Input: part model. Units: mm. Frame: model coordinates. A direction names the side the tool comes from. Coordinates: 2 decimals unless noted, no trailing zeros. Write each loop counter-clockwise with the first axis right and the second up, starting at its lowest first coordinate (ties: lowest second). Pieces come first, ordered by that corner, then holes. Notation, with made-up numbers: (82.25, 18.25) - (109.25, 18.25) arc R5 ccw to (109.25, 27.25) - close; hole circle Ø7 at (17, -23.5). An arc over 180 degrees is marked (long way). Put each result on its own line as item: value. Start each with the question number.
1. Cut plane B-B, the plane z = -3.25. Return loops of the section in (x, y).
2. Line query: line 1 (Z direction, x = 9, y = 6); line 2 (X direction, y = 0.25, z = -2.5); line 3 (Y direction, x = 8, z = 2.5). Output: solid intervals per line, ascending.
3. Access query for faces 1 (the cylindrical face through (10.29, -0.97, -8.66)), 2 (the cylindrical face through (-5.587, -0.975, 8.713)), 3 (the cylindrical face through (-0.09, -6.79, -5.79)), 4 (the flat face through (0, 0, -4.7)). Directions: +Z, -Z, +X, -X, +Y, -Y. A direction counts if a zero-diameter tool reaches every point of the face in a straight line with its end or side. Return the directions, or none.
4. Cut plane A-A, the plane x = 2.5. Return loops of the section in (y, z), and give its area (3 significant figures).
5. Cut plane C-C, the plane y = -6.25. Return loops of the section in (x, z).
6. Pull-direction query (X, two-part tool) for faces 5 (the cylindrical face through (0.09, 6.79, -5.79)), 6 (the flat face through (-8, 0, -10.9)); classes: released by +X, released by -X, zero draft, split by the parting line, or undercut.
7. Cut plane D-D, the plane y = 3.75. Return loops of the section in (x, z), and give its area (3 significant figures).
8. Pin query (flat end, axial travel): pin 1 (2 mm diameter, centred on y = -3.5, z = -3, fed in from -X); pin 2 (1.5 mm diameter, centred on x = 2.5, y = -0.5, fed in from -Z); pin 3 (3 mm diameter, centred on x = -12, z = -1, fed in from +Y). Return the tip coordinate at first contact, or that it passes through.
from build123d import *

# Parameters (mm, degrees)
SKETCH_2_R        = 5.08
EXTRUDE_1_DEPTH   = 4.7
EXTRUDE_1_2_DEPTH = 4.7
EXTRUDE_2_DEPTH   = 2.22
SKETCH_4_R        = 2.545
EXTRUDE_3_DEPTH   = 10.9
CHAMFER_1_SIZE    = 0.444


with BuildPart() as part:
    # Sketch 2 → Extrude 1 (new, symmetric)
    with BuildSketch(Plane.XY):
        with Locations((7.9375, 0)):
            Circle(SKETCH_2_R)
    extrude(amount=EXTRUDE_1_DEPTH, both=True)



with BuildPart() as body_2:
    # Sketch 2 → Extrude 1 2 (new, symmetric)
    with BuildSketch(Plane.XY):
        with Locations((-7.9375, 0)):
            Circle(SKETCH_2_R)
    extrude(amount=EXTRUDE_1_2_DEPTH, both=True)


with BuildPart() as part_1:
    add(part.part)

    add(body_2.part)  # Extrude 2 merges body 2
    # Sketch 3 → Extrude 2 (add)
    with BuildSketch(Plane.XY.offset(4.7)):
        with BuildLine():
            ThreePointArc((-6.515962535, 7.409875588), (-15.4825, 0), (-6.515962535, -7.409875588))
            ThreePointArc((-6.515962535, -7.409875588), (0, -6.7905), (6.515962535, -7.409875588))
            ThreePointArc((6.515962535, -7.409875588), (15.4825, 0), (6.515962535, 7.409875588))
            ThreePointArc((6.515962535, 7.409875588), (0, 6.7905), (-6.515962535, 7.409875588))
        make_face()
    extrude_2 = extrude(amount=EXTRUDE_2_DEPTH)

    # Mirror 1: Extrude 2 across plane
    add(extrude_2.mirror(Plane.XY))

    # Sketch 4 → Extrude 3 (add, symmetric)
    with BuildSketch(Plane.XY):
        with Locations((7.9375, 0)):
            Circle(SKETCH_4_R)
        with Locations((-7.9375, 0)):
            Circle(SKETCH_4_R)
    extrude(amount=EXTRUDE_3_DEPTH, both=True)

    # Chamfer 1
    chamfer_1_edges = [part_1.edges().sort_by_distance(p)[0] for p in [
        (5.3925, 0, -10.9),
        (5.3925, 0, 10.9),
        (-10.4825, 0, -10.9),
        (-10.4825, 0, 10.9),
    ]]
    chamfer(chamfer_1_edges, length=CHAMFER_1_SIZE)


solid = part_1.part
Report:
1. outline: circle Ø10.16 at (-7.94, 0); circle Ø10.16 at (7.94, 0)
2. line 1: z = -6.92 to -4.7, 4.7 to 6.92
2. line 2: x = -13.01 to -2.86, 2.86 to 13.01
2. line 3: y = -5.08 to 5.08
3. face 1: -Z
3. face 2: +Z
3. face 3: +Z, -Z, -Y
3. face 4: none
4. outline: (-6.88, -6.92) - (6.88, -6.92) - (6.88, -4.7) - (-6.88, -4.7) - close; (-6.88, 4.7) - (6.88, 4.7) - (6.88, 6.92) - (-6.88, 6.92) - close
4. area: 61.1 mm^2
5. outline: (-12.16, -6.92) - (12.16, -6.92) - (12.16, -4.7) - (-12.16, -4.7) - close; (-12.16, 4.7) - (12.16, 4.7) - (12.16, 6.92) - (-12.16, 6.92) - close
6. face 5: undercut
6. face 6: zero draft
7. outline: (-14.48, -6.92) - (14.48, -6.92) - (14.48, -4.7) - (11.36, -4.7) - (11.36, 4.7) - (14.48, 4.7) - (14.48, 6.92) - (-14.48, 6.92) - (-14.48, 4.7) - (-11.36, 4.7) - (-11.36, -4.7) - (-14.48, -4.7) - close; hole (-4.51, -4.7) - (4.51, -4.7) - (4.51, 4.7) - (-4.51, 4.7) - close
7. area: 257 mm^2
8. pin 1: stops at x = -12.36
8. pin 2: stops at z = -6.92
8. pin 3: stops at y = 4.39
